Source: CAD feature listing. Evaluate the final solid. Frame: model axes, mm. A direction names the side the tool comes from. Give positions to 0.01 mm unless a question says otherwise; leave off trailing zeros. Loops run counter-clockwise (first coordinate to the right, second up) from the corner with the lowest first, then second, coordinate; pieces in that order, holes last. Notation, with made-up numbers: (41.25, 3.5) - (94.25, 3.5) arc R25 ccw to (94.25, 24.5) - close; hole circle Ø1 at (13, 48). An arc over 180 degrees is marked (long way). Put each result on its own line as item: value.
```python
from build123d import *
from build123d.topology import SkipClean

# Parameters (mm, degrees)
SKETCH_1_R             = 6.25
EXTRUDE_1_DEPTH        = 28
SKETCH_2_R             = 10.85
EXTRUDE_2_DEPTH        = 4.5
CUT_EXTRUDE_START      = -12
CUT_EXTRUDE_1_DEPTH    = 12
SKETCH_4_R             = 4
CUT_EXTRUDE_2_DEPTH    = 42.744550687
HOLE_WIZARD_M8_1_D     = 6.8
HOLE_WIZARD_M8_1_DEPTH = 12
HOLE_WIZARD_M8_1_TIP   = 2.042926105
SKETCH_8_R             = 6
SKETCH_8_R_2           = 4
EXTRUDE_3_DEPTH        = 5.95


with BuildPart() as part:
    # 草图1 → 凸台-拉伸1 (new body)
    with BuildSketch(Plane.XY):
        Circle(SKETCH_1_R)
    extrude(amount=EXTRUDE_1_DEPTH)

    # 草图2 → 凸台-拉伸2 (add, symmetric)
    with BuildSketch(Plane(origin=(0, 0, 0), x_dir=(1, 0, 0), z_dir=(0, 1, 0))):
        with Locations((0, -28)):
            Circle(SKETCH_2_R)
    extrude(amount=EXTRUDE_2_DEPTH, both=True)

    # 草图3 → 切除-拉伸1 (cut)
    with BuildSketch(Plane.XY.offset(28).offset(CUT_EXTRUDE_START)):
        with BuildLine():
            Line((4.337337893, -4.5), (-4.337337893, -4.5))
            ThreePointArc((-4.337337893, -4.5), (0, -6.25), (4.337337893, -4.5))
        make_face()
        with BuildLine():
            Line((-4.337337893, 4.5), (4.337337893, 4.5))
            ThreePointArc((4.337337893, 4.5), (0, 6.25), (-4.337337893, 4.5))
        make_face()
    extrude(amount=CUT_EXTRUDE_1_DEPTH, mode=Mode.SUBTRACT)

    # 草图4 → 切除-拉伸2 (cut, through all)
    with BuildSketch(Plane.XZ.offset(4.5)):
        with Locations(Location((0, 28, 0), (0, 0, 270))):
            Circle(SKETCH_4_R)
    extrude(amount=-CUT_EXTRUDE_2_DEPTH, mode=Mode.SUBTRACT)

    # M8 螺纹孔1
    with Locations(Plane(origin=(0, 0, 0), x_dir=(-1, 0, 0), z_dir=(0, 0, -1))):
        with Locations((0, 0)):
            Hole(HOLE_WIZARD_M8_1_D / 2, depth=HOLE_WIZARD_M8_1_DEPTH)
            with Locations((0, 0, -(HOLE_WIZARD_M8_1_DEPTH + HOLE_WIZARD_M8_1_TIP / 2))):  # 118° drill point
                Cone(0, HOLE_WIZARD_M8_1_D / 2, HOLE_WIZARD_M8_1_TIP, mode=Mode.SUBTRACT)

    # 草图8 → 凸台-拉伸3 (add, symmetric)
    with SkipClean():  # the faces are left unmerged after this step: merging them gives an invalid solid
        with BuildSketch(Plane(origin=(0, 0, 0), x_dir=(1, 0, 0), z_dir=(0, 1, 0))):
            with Locations(Location((0, -28, 0), (0, 0, 270))):
                Circle(SKETCH_8_R)
            with Locations(Location((0, -28, 0), (0, 0, 270))):
                Circle(SKETCH_8_R_2, mode=Mode.SUBTRACT)
        extrude(amount=EXTRUDE_3_DEPTH, both=True)


solid = part.part
```
1) Section query A-A, the plane z = 28. Output: boundary loops of the cut face in (x, y), plus the area to 3 significant figures.
Check result:
outline: (-10.85, -4.5) - (-6, -4.5) - (-6, -5.95) - (-4, -5.95) - (-4, 5.95) - (-6, 5.95) - (-6, 4.5) - (-10.85, 4.5) - close; (4, -5.95) - (6, -5.95) - (6, -4.5) - (10.85, -4.5) - (10.85, 4.5) - (6, 4.5) - (6, 5.95) - (4, 5.95) - close
area: 135 mm²
2) Access query for faces 1 (the flat face through (1.42, -5.95, 31.92)), 2 (the flat face through (0, 5, 16)), 3 (the flat face through (2, -4.5, 22)), 4 (the cylindrical face through (-0.74, -3.32, 6.08)), 5 (the flat face through (2, 4.5, 22)). Directions: +Z, -Z, +X, -X, +Y, -Y. A direction counts if a zero-diameter tool reaches every point of the face in a straight line with its end or side. Return the directions, or none.
Check result:
face 1: +Z, +X, -X, -Y
face 2: +X, -X, +Y
face 3: -Y
face 4: -Z
face 5: +Y
3) Mould query, pull axis Z, two halves, no side actions, for faces 6 (the cylindrical face through (-0.415, 0.063, 38.842)), 7 (the flat face through (0, -5, 16)), 8 (the flat face through (3, -3, 0)), 9 (the cylindrical face through (-6.244, 0.275, 9.432)). Classes: pulls with the +Z half, pulls with the -Z half, needs draft (parallel to the pull), parting line crosses it, or undercut.
Check result:
face 6: parting line crosses it
face 7: undercut
face 8: pulls with the -Z half
face 9: needs draft
4) Material intervals for line 1 along X through (y, z) = (-5.4, 28); line 2 along Y through (x, z) = (0, 7); line 3 along X through (y, z) = (0, 14.5), sorted ascending. Write a range as [from, to].
Check result:
line 1: [-6, -4], [4, 6]
line 2: [-6.25, -3.4], [3.4, 6.25]
line 3: [-6.25, 6.25]
5) Section query B-B, the plane z = 3.5. Output: boundary loops of the cut face in (x, y), plus the area to 3 significant figures.
Check result:
outline: circle Ø12.5 at (0, 0); hole circle Ø6.8 at (0, 0)
area: 86.4 mm²
6) Section query D-D, the plane x = 8.5. Output: boundary loops of the cut face in (y, z), plus the area to 3 significant figures.
Check result:
outline: (-4.5, 21.26) - (4.5, 21.26) - (4.5, 34.74) - (-4.5, 34.74) - close
area: 121 mm²
7) Section query C-C, the plane z = 33.5. Output: boundary loops of the cut face in (x, y).
Check result:
outline: (-9.35, -4.5) - (-2.4, -4.5) - (-2.4, -5.95) - (2.4, -5.95) - (2.4, -4.5) - (9.35, -4.5) - (9.35, 4.5) - (2.4, 4.5) - (2.4, 5.95) - (-2.4, 5.95) - (-2.4, 4.5) - (-9.35, 4.5) - close
8) Pin query (flat end, axial travel): P1, Ø3.5, axis at x = 1, z = 29, coming from the +Y side; P2, Ø3, axis at y = -0.5, z = 26, coming from the -X side; P3, Ø1, axis at x = 7, y = -1, coming from the +Z side; P4, Ø1, axis at x = 2, z = 5.5, coming from the +Y side. Return the tip coordinate at first contact, or that it passes through.
Check result:
P1: through
P2: x = -10.84
P3: z = 36.69
P4: y = 6.07
